Print and shaded views of the part. All mm, measured from the part's lowest x, y and z. A direction names the side the tool comes from. Give positions to 0.01 mm unless a question says otherwise; leave off trailing zeros. Write each loop counter-clockwise with the first axis right and the second up, starting at its lowest first coordinate (ties: lowest second). Pieces come first, ordered by that corner, then holes. Notation, with made-up numbers: M -10,45.5 L 21,45.5 A12 cw 21,59.5 Z; hole C 61,74 d9. An arc over 180 degrees is marked long. One line per question, with ' | ' between items. Start each with the question number.
1. Cut at C-C, the plane x = 78.5. Write the cut outline in (y, z).
2. Cut at A-A, the plane x = 45. Count the separate pieces of the cut face and the enclosed holes in it, then the cut area to 3 significant figures.
3. Flat gauge pins, fed straight in: pin 1 (5 mm diameter, centred on y = 35, z = 17, fed in from +X); pin 2 (24 mm diameter, centred on x = 45, y = 45, fed in from +Z); pin 3 (6 mm diameter, centred on y = 52, z = 62.5, fed in from +X); pin 4 (5 mm diameter, centred on x = 55, z = 50.5, fed in from -Y). Where does each tip first touch, or does it go through?
4. Cut at B-B, the plane y = 79. Write the cut outline in (x, z), then the cut area to 3 significant figures.
5. Cut at D-D, the plane z = 49.5. Write the cut outline in (x, y).
6. Which spindle directions (+Z, -Z, +X, -X, +Y, -Y) get a long thin tool onto all of the face, cutting with end or side? Do the marked faces 1, 2 and 3. Say none if no direction does.
7. Pull direction Z, two halves, no side cores. Call the marked faces 4, 5 and 6: released by +Z, released by -Z, zero draft, split by the parting line, or undercut.
8. Wall check: L1, parallel to Y at x = 45, z = 8.5; L2, parallel to Z at x = 63, y = 61; L3, parallel to Y at x = 45, z = 16. Give the ranges that are in metal, low to high.
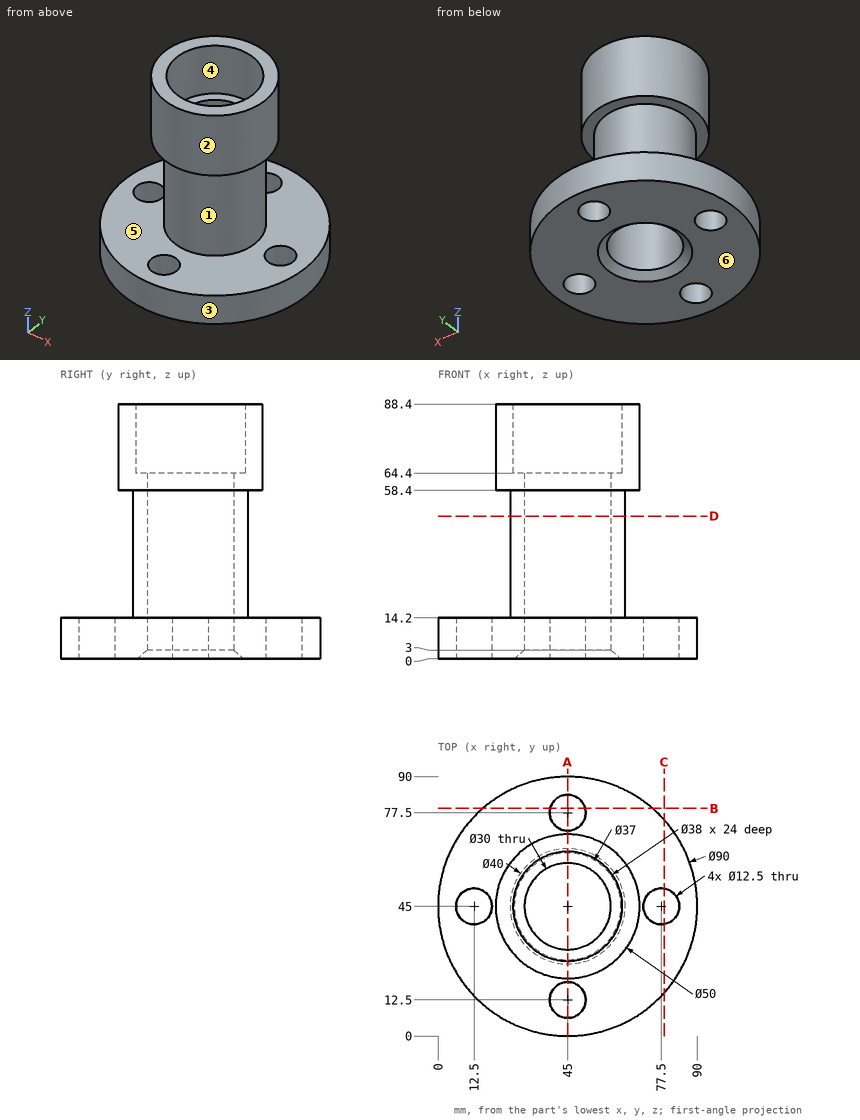
Here are the results:
1) outline: M 14.95,0 L 38.83,0 L 38.83,14.2 L 14.95,14.2 Z; M 51.17,0 L 75.05,0 L 75.05,14.2 L 51.17,14.2 Z
2) separate pieces: 4 | enclosed holes: 0 | area: 1,340 mm^2
3) pin 1: x = 63.54 | pin 2: through | pin 3: x = 69.68 | pin 4: y = 26.46
4) outline: M 15.52,0 L 38.93,0 L 38.93,14.2 L 15.52,14.2 Z; M 51.07,0 L 74.48,0 L 74.48,14.2 L 51.07,14.2 Z | area: 665 mm^2
5) outline: C 45,45 d40; hole C 45,45 d30
6) face 1: none | face 2: +Z | face 3: +Z, -Z
7) face 4: zero draft | face 5: undercut | face 6: released by -Z
8) L1: 0 to 6.25, 18.75 to 30, 60 to 71.25, 83.75 to 90 | L2: 0 to 14.2, 58.4 to 88.4 | L3: 25 to 30, 60 to 65
